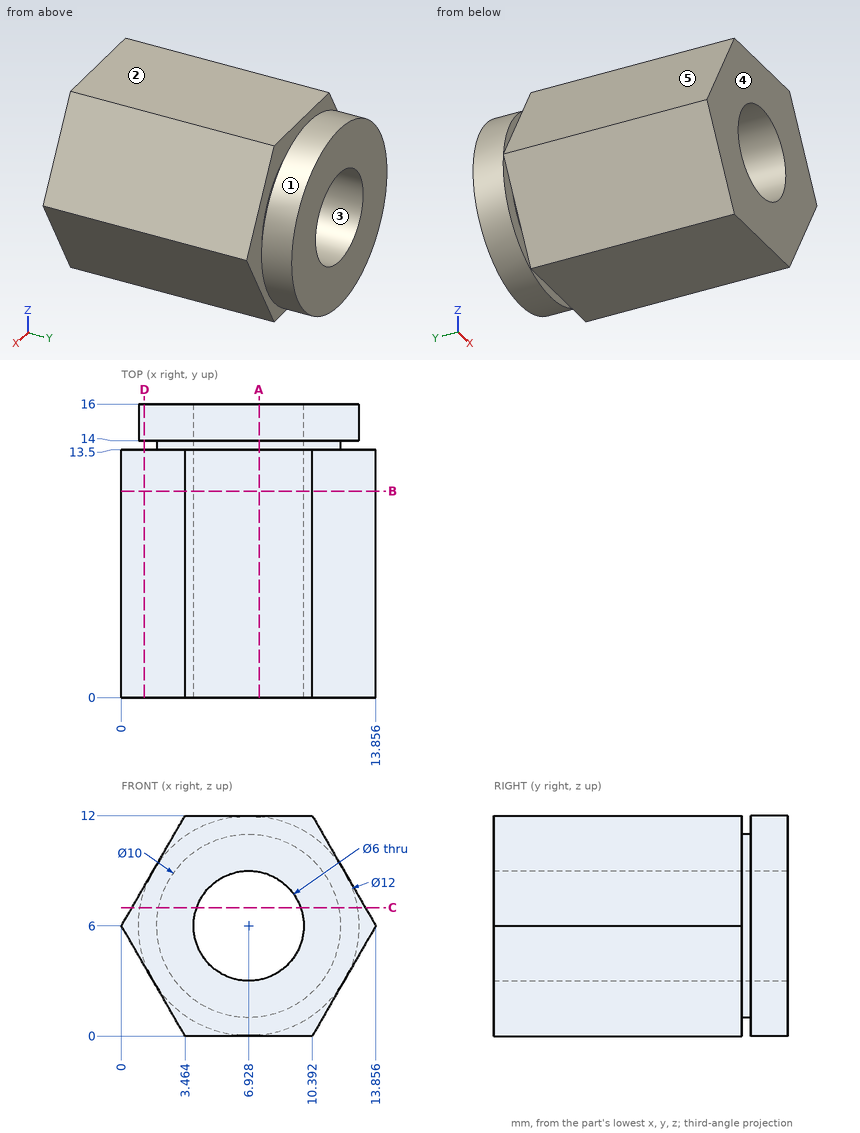
Check sheet for the drawn part. Datum: minimum x, y, z corner. Units: mm. A direction names the side the tool comes from. Round coordinates to 2 decimals unless told otherwise and drop trailing zeros. Order: outer loops, then holes, each group sorted by start corner. A loop starts at its lowest first (then second) coordinate and runs counter-clockwise, first axis right, second up.
1) Mould release check, pull along X, two halves, no side actions. Record for the marked faces 3, 4 and 5: +X half, -X half, draft (parallel to the pull), parting line (faces both ways), or undercut.
2) Section check A-A (x = 7.5). Record the boundary of the cut face in (y, z) (1 decimal).
3) Scan lines: line 1 (Y direction, x = 12.5, z = 7.5); line 2 (Z direction, x = 7, y = 2); line 3 (Z direction, x = 8, y = 12.75). Record each from-to range of solid material in increasing order.
4) Section check C-C (z = 7). Record the boundary of the cut face in (x, y) (1 decimal).
5) Section check B-B (y = 11.25). Record the boundary of the cut face in (x, z).
6) Section check D-D (x = 1.25). Record the boundary of the cut face in (y, z) (1 decimal).
7) Go/stop test with a flat-tipped pin: pin 1 Ø2 at (y, z) = (2.5, 10.5) entering from -X. Record where the tip stops, or that it passes through.
8) Tool access check on the marked faces 1 and 2. Record the directions out of +Z, -Z, +X, -X, +Y, -Y that give a thin tool (end or side, any length) a straight path to the whole face; none if there is none.
Result:
1. face 3: undercut
1. face 4: draft
1. face 5: -X half
2. outline: (0, 0) - (13.5, 0) - (13.5, 1) - (14, 1) - (14, 0) - (16, 0) - (16, 3.1) - (0, 3.1) - close; (0, 8.9) - (16, 8.9) - (16, 12) - (14, 12) - (14, 11) - (13.5, 11) - (13.5, 12) - (0, 12) - close
3. line 1: y = 0 to 13.5, 14 to 16
3. line 2: z = 0 to 3, 9 to 12
3. line 3: z = 0 to 3.2, 8.8 to 12
4. outline: (0.6, 0) - (4.1, 0) - (4.1, 16) - (1, 16) - (1, 14) - (2, 14) - (2, 13.5) - (0.6, 13.5) - close; (9.8, 0) - (13.3, 0) - (13.3, 13.5) - (11.8, 13.5) - (11.8, 14) - (12.8, 14) - (12.8, 16) - (9.8, 16) - close
5. outline: (0, 6) - (3.46, 0) - (10.39, 0) - (13.86, 6) - (10.39, 12) - (3.46, 12) - close; hole circle Ø6 at (6.93, 6)
6. outline: (0, 3.8) - (13.5, 3.8) - (13.5, 8.2) - (0, 8.2) - close; (14, 4.1) - (16, 4.1) - (16, 7.9) - (14, 7.9) - close
7. pin 1: stops at x = 2.02
8. face 1: +Y
8. face 2: +Z, +X, -X, +Y, -Y
